Here's how the part is built. I have some questions about the finished solid (model axes, mm). A direction names the side the tool comes from. Coordinates: 2 decimals unless noted, no trailing zeros. Order: outer loops, then holes, each group sorted by start corner. A loop starts at its lowest first (then second) coordinate and runs counter-clockwise, first axis right, second up. Notation, with made-up numbers: M 57.5,89 L 108.5,89 A18 cw 108.5,102 Z; hole C 38.5,2.5 d8. An arc over 180 degrees is marked long. One line per question, with ' | ' between items. Start each with the question number.
```python
from build123d import *

# Parameters (mm, degrees)
CLEVIS_BODY_PROFILE_R   = 11
CLEVIS_BODY_PROFILE_R_2 = 2.5
CLEVIS_BODY_DEPTH       = 25
CLEVIS_SLOT_SKETCH_W    = 90.532278548
CLEVIS_SLOT_SKETCH_H    = 30
CLEVIS_SLOT_30MM_DEPTH  = 86.732140997
EAR_SIDE_RELIEF_DEPTH   = 4
SLOT_FILLET_R1_5_R      = 1.5


with BuildPart() as part:
    # Clevis Body Profile → Clevis Body (new, symmetric)
    with BuildSketch(Plane.XY):
        with BuildLine():
            Line((-65, 25), (11.583123952, 25))
            ThreePointArc((11.583123952, 25), (25, 0), (11.583123952, -25))
            Line((11.583123952, -25), (-65, -25))
            Line((-65, -25), (-65, 25))
        make_face()
        Circle(CLEVIS_BODY_PROFILE_R, mode=Mode.SUBTRACT)
        with Locations((-40, -7.5)):
            Circle(CLEVIS_BODY_PROFILE_R_2, mode=Mode.SUBTRACT)
    extrude(amount=CLEVIS_BODY_DEPTH, both=True)

    # Clevis Slot Sketch → Clevis Slot 30mm (cut, through all)
    with BuildSketch(Plane(origin=(0, 25, 0), x_dir=(1, 0, 0), z_dir=(0, 1, 0))):
        with Locations((-4.733860726, 0)):
            Rectangle(CLEVIS_SLOT_SKETCH_W, CLEVIS_SLOT_SKETCH_H)
    extrude(amount=-CLEVIS_SLOT_30MM_DEPTH, mode=Mode.SUBTRACT)

    # Ear Side Relief Sketch → Ear Side Relief (cut)
    with BuildSketch(Plane.XY.offset(25)):
        with BuildLine():
            Line((-39, 25), (-20.801488287, -25))
            Line((-20.801488287, -25), (11.583123952, -25))
            ThreePointArc((11.583123952, -25), (25, 0), (11.583123952, 25))
            Line((11.583123952, 25), (-39, 25))
        make_face()
    ear_side_relief = extrude(amount=-EAR_SIDE_RELIEF_DEPTH, mode=Mode.SUBTRACT)

    # Ear Side Relief Mirror: Ear Side Relief across plane
    add(ear_side_relief.mirror(Plane.XY), mode=Mode.SUBTRACT)

    # Slot Fillet R1.5
    slot_fillet_r1_5_edges = [part.edges().sort_by_distance(p)[0] for p in [
        (-50, 0, -15),
        (-50, 0, 15),
    ]]
    fillet(slot_fillet_r1_5_edges, radius=SLOT_FILLET_R1_5_R)

    # Sketch4 → Pin Bore Ø20 CBore Ø35 (revolve, cut)
    with BuildSketch(Plane(origin=(-65, 0, 0), x_dir=(0, 0, 1), z_dir=(0, 1, 0))):
        Polygon((0, 0), (0, 99.718353376), (10, 99.718353376), (10, 2), (17.5, 2), (17.5, 0), align=None)
    revolve(axis=Axis((45, 0, 0), (-1, 0, 0)), mode=Mode.SUBTRACT)


solid = part.part
```
1. Which directions (+Z, -Z, +X, -X, +Y, -Y) give clear straight access to the entire face, cutting with the end or side of a thin tool? Please do faces 4 (the face through (-30.03, 0.35, -23.03)), 5 (the face through (-12, 0, 15)), 6 (the face through (-30.03, 0.35, 23.03)), 7 (the face through (-63, -8, -8)), 8 (the face through (-37.69, -8.46, -20.07)).
2. Imagine slicing it at C-C (z = -3). List the corners of the cut face in (x, y) for me, then the cut area to 3 significant figures.
3. We'd pull the mould along Y, two halves only. Please class faces 1 (the face through (-64.014, -10.648, -13.887)), 2 (the face through (-52, -25, 0)), 3 (the face through (-15, 0, 21)): released by +Y, released by -Y, zero draft, split by the parting line, or undercut.
4. Imagine slicing it at A-A (x = 0). List the corners of the cut face in (y, z) for me.
5. Imagine slicing it at B-B (y = 0). Count the separate pieces of the cut face and the enclosed holes in it, then the cut area to 3 significant figures.
6. I need wall thicknesses on line 1 (Z direction, x = -39, y = 8); line 2 (Z direction, x = 16, y = -5); line 3 (Y direction, x = -58.75, z = 0). Which ranges of each line are inside material? Lowest first, please.
7. Imagine slicing it at D-D (x = -28). List the corners of the cut face in (y, z) for me.
8. Will these pins go through, and if not, where does the flat tip stop? pin 1 (3 mm diameter, centred on x = 2.5, y = 17, fed in from +Z); pin 2 (3 mm diameter, centred on x = 15.5, y = -18.5, fed in from -Z); pin 3 (10 mm diameter, centred on y = 14.5, z = 16.5, fed in from +X).
Entries:
1) face 4: -Z, +X, +Y | face 5: +X, +Y, -Y | face 6: +Z, +X, +Y | face 7: -X | face 8: +Z, -Z
2) outline: M -65,-25 L -50,-25 L -50,-9.54 L -63,-9.54 L -63,-17.24 L -65,-17.24 Z; M -65,17.24 L -63,17.24 L -63,9.54 L -50,9.54 L -50,25 L -65,25 Z | area: 433 mm²
3) face 1: undercut | face 2: released by -Y | face 3: zero draft
4) outline: M -25,-21 L -11,-21 L -11,-15 L -25,-15 Z; M -25,15 L -11,15 L -11,21 L -25,21 Z; M 11,-21 L 25,-21 L 25,-15 L 11,-15 Z; M 11,15 L 25,15 L 25,21 L 11,21 Z
5) separate pieces: 4 | enclosed holes: 0 | area: 1,220 mm²
6) line 1: -25 to -15, 15 to 25 | line 2: -21 to -15, 15 to 21 | line 3: -25 to -10, 10 to 25
7) outline: M -25,-25 L -5.22,-25 L -5.22,-21 L 25,-21 L 25,-15 L -25,-15 Z; M -25,15 L 25,15 L 25,21 L -5.22,21 L -5.22,25 L -25,25 Z
8) pin 1: z = 21 | pin 2: z = -21 | pin 3: x = 23.46
